from build123d import *

# Parameters (mm, degrees)
BOSS_EXTRUDE1_DEPTH = 9
BOSS_EXTRUDE2_START = 39
SKETCH5_R           = 10
BOSS_EXTRUDE2_DEPTH = 15
CHAMFER1_SIZE       = 1


with BuildPart() as part:
    # Sketch1 → Revolve1 (revolve)
    with BuildSketch(Plane.XY, mode=Mode.PRIVATE) as revolve1_sk:
        Polygon((15, 0), (40, 0), (40, 9.5), (39.5, 10), (40, 10.5), (40, 20), (22, 20), (21, 31), (10, 31), (10, 181), (0, 181), (0, 15), (14, 15), align=None)
    revolve(revolve1_sk.sketch.rotate(Axis((0, 181, 0), (0, -1, 0)), 180), axis=Axis((0, 181, 0), (0, -1, 0)))

    # Sketch2 → Boss-Extrude1 (add)
    with BuildSketch(Plane(origin=(0, 31, 0), x_dir=(1, 0, 0), z_dir=(0, 1, 0))):
        Polygon((12, 6.92820323), (0, 13.856406461), (-12, 6.92820323), (-12, -6.92820323), (0, -13.856406461), (12, -6.92820323), align=None)
    extrude(amount=BOSS_EXTRUDE1_DEPTH)

    # Sketch3 → Cut-Revolve1 (revolve, cut)
    with BuildSketch(Plane(origin=(0, 0, 0), x_dir=(0, 0, -1), z_dir=(1, 0, 0))):
        Polygon((12.356406461, 31), (13.856406461, 31.866025404), (13.856406461, 31), align=None)
        Polygon((13.856406461, 39.422649731), (12.856406461, 40), (13.856406461, 40), align=None)
    revolve(axis=Axis((0, 181, 0), (0, 1, 0)), mode=Mode.SUBTRACT)

    # Sketch5 → Boss-Extrude2 (add)
    with BuildSketch(Plane(origin=(0, 41, 0), x_dir=(-1, 0, 0), z_dir=(0, 1, 0)).offset(BOSS_EXTRUDE2_START)):
        Polygon((0, 19.225763964), (-16.65, 9.612881982), (-16.65, -9.612881982), (0, -19.225763964), (16.65, -9.612881982), (16.65, 9.612881982), align=None)
        with Locations(Location((0, 0, 0), (0, 0, 90))):
            Circle(SKETCH5_R, mode=Mode.SUBTRACT)
    extrude(amount=-BOSS_EXTRUDE2_DEPTH)

    # Sketch7 → Cut-Revolve3 (revolve, cut)
    with BuildSketch(Plane(origin=(0, 0, 0), x_dir=(0, 0, -1), z_dir=(1, 0, 0)), mode=Mode.PRIVATE) as cut_revolve3_sk:
        Polygon((16.525763964, 80), (19.225763964, 77.3), (19.225763964, 80), align=None)
        Polygon((16.525763964, 41), (19.225763964, 43.7), (19.225763964, 41), align=None)
    revolve(cut_revolve3_sk.sketch.rotate(Axis((0, 181, 0), (0, 1, 0)), 180), axis=Axis((0, 181, 0), (0, 1, 0)), mode=Mode.SUBTRACT)

    # Chamfer1
    chamfer1_edges = [part.edges().sort_by_distance(p)[0] for p in [
        (10, 181, 0),
    ]]
    chamfer(chamfer1_edges, length=CHAMFER1_SIZE)


solid = part.part
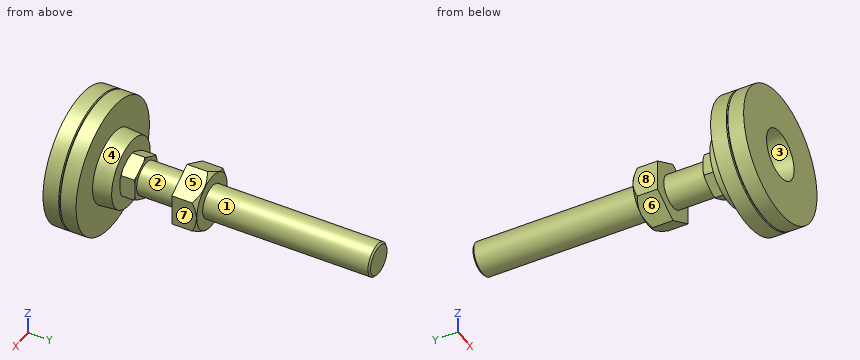
Model file for the job. Use its own axes, mm. Face numbers are marked on the shaded views. A direction names the side the tool comes from. Coordinates: 2 decimals unless noted, no trailing zeros. Order: outer loops, then holes, each group sorted by start corner. A loop starts at its lowest first (then second) coordinate and runs counter-clockwise, first axis right, second up. Notation, with made-up numbers: (7, 55.25) -> (14, 55.25) arc R11 cw to (14, 69.25) -> close; hole circle Ø3 at (51, -8.5). An arc over 180 degrees is marked (long way). Return JSON: item names as keys, results as strings. Group by question number.
Item 1: Pull direction Y, two halves, no side cores. Call the marked faces 1, 2, 3 and 4: pulls with the +Y half, pulls with the -Y half, needs draft (parallel to the pull), parting line crosses it, or undercut.
Item 2: Tool access for the marked faces 5, 6, 7 and 8: list every direction of +Z, -Z, +X, -X, +Y, -Y with a clear straight run to the whole face (end or side of a thin tool).
Item 3: Saw through at A-A on y = 73. Write the cut outline in (x, z).
Item 4: Wall check: line 1 along Y through (x, z) = (10, -9); line 2 along Y through (x, z) = (-4, 26.5); line 3 along Y through (x, z) = (-2, 0). Give the ranges that are in metal, low to high. Write a range as [from, to].
Item 5: Flat gauge pins, fed straight in: P1, Ø10, axis at x = 4, z = 0.5, coming from the -Y side; P2, Ø7, axis at y = 37, z = 2.5, coming from the +X side; P3, Ø8, axis at x = 13, y = 101, coming from the -Z side; P4, Ø12, axis at y = 63, z = -28.5, coming from the -X side. Where does each tip first touch, or does it go through?
Values found:
{
 "1": {"face 1": "needs draft", "face 2": "undercut", "face 3": "pulls with the -Y half", "face 4": "pulls with the +Y half"},
 "2": {"face 5": "+Z, +X, +Y", "face 6": "-Z, -X, +Y", "face 7": "+Z, -Z, +X, +Y", "face 8": "+Z, -Z, -X, +Y"},
 "3": {"outline": "(-16.65, -9.61) -> (0, -19.23) -> (16.65, -9.61) -> (16.65, 9.61) -> (0, 19.23) -> (-16.65, 9.61) -> close"},
 "4": {"line 1": "y = [15, 31], [65, 80]", "line 2": "y = [0, 20]", "line 3": "y = [15, 181]"},
 "5": {"P1": "stops at y = 15", "P2": "stops at x = 12", "P3": "stops at z = -4.36", "P4": "passes through"}
}
